Here's the drawing with two shaded views (mm, measured from the low corner). I have some questions. Round coordinates to 2 decimals unless told otherwise and drop trailing zeros. Write each loop counter-clockwise with the first axis right and the second up, starting at its lowest first coordinate (ties: lowest second). Pieces come first, ordered by that corner, then holes. Notation, with made-up numbers: M 87,14.5 L 94,14.5 A21 ccw 94,27.5 Z; hole C -23.75,69 d6. An arc over 180 degrees is marked long. Use one line per item in the form item = value. Start each with the question number.
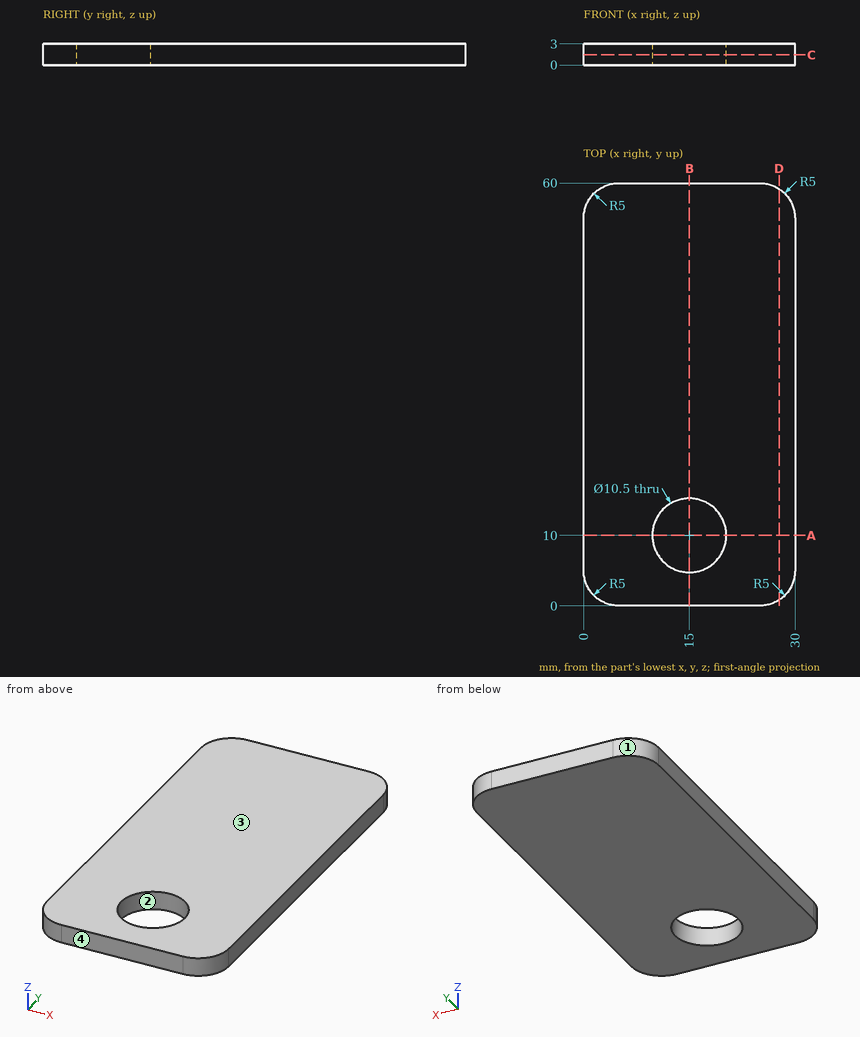
1. If we section it at B-B (x = 15): List the corners of the cut face in (y, z) for me.
2. If we section it at D-D (x = 27.75): List the corners of the cut face in (y, z) for me, and give its area (3 significant figures).
3. If we mould it in two halves opening along Y, with no side actions, what happens to the marked faces 1, 2, 3 and 4? For each: pulls with the +Y half, pulls with the -Y half, needs draft (parallel to the pull), parting line crosses it, or undercut.
4. If we section it at A-A (y = 10): List the corners of the cut face in (x, z) for me.
5. Please list where these lines run through material, in increasing order: line 1 along Y through (x, z) = (15, 1.9); line 2 along Y through (x, z) = (11.25, 0.4); line 3 along X through (y, z) = (12, 2.15).
6. If we section it at C-C (z = 1.45): List the corners of the cut face in (x, y) for me, and give its area (3 significant figures).
Model answer:
q1.outline = M 0,0 L 4.75,0 L 4.75,3 L 0,3 Z; M 15.25,0 L 60,0 L 60,3 L 15.25,3 Z
q2.outline = M 0.82,0 L 59.18,0 L 59.18,3 L 0.82,3 Z
q2.area = 175 mm2
q3.face_1 = pulls with the +Y half
q3.face_2 = undercut
q3.face_3 = needs draft
q3.face_4 = pulls with the -Y half
q4.outline = M 0,0 L 9.75,0 L 9.75,3 L 0,3 Z; M 20.25,0 L 30,0 L 30,3 L 20.25,3 Z
q5.line_1 = 0 to 4.75, 15.25 to 60
q5.line_2 = 0 to 6.33, 13.67 to 60
q5.line_3 = 0 to 10.15, 19.85 to 30
q6.outline = M 0,5 A5 ccw 5,0 L 25,0 A5 ccw 30,5 L 30,55 A5 ccw 25,60 L 5,60 A5 ccw 0,55 Z; hole C 15,10 d10.5
q6.area = 1,690 mm2
